from build123d import *

# Parameters (mm, degrees)
BOSS_EXTRUDE1_DEPTH = 5
SKETCH2_W           = 20
SKETCH2_H           = 6
SKETCH2_R           = 1.5
BOSS_EXTRUDE2_DEPTH = 2
SKETCH3_W           = 60
SKETCH3_H           = 6
BOSS_EXTRUDE3_DEPTH = 2


with BuildPart() as part:
    # Sketch1 → Boss-Extrude1 (new, symmetric)
    with BuildSketch(Plane.XY):
        Polygon((-14.216216216, 5.673798061), (-14.216216216, 15.673798061), (-16.216216216, 15.673798061), (-16.216216216, 3.673798061), (3.783783784, 3.673798061), (3.783783784, -6.326201939), (5.783783784, -6.326201939), (5.783783784, 5.673798061), align=None)
    extrude(amount=BOSS_EXTRUDE1_DEPTH, both=True)

    # Sketch2 → Boss-Extrude2 (add)
    with BuildSketch(Plane(origin=(5.783783784, 0, 0), x_dir=(0, 0, -1), z_dir=(1, 0, 0))):
        with Locations((0, -3.326201939)):
            Rectangle(SKETCH2_W, SKETCH2_H)
        with Locations((-7, -3.326201939)):
            Circle(SKETCH2_R, mode=Mode.SUBTRACT)
        with Locations((7, -3.326201939)):
            Circle(SKETCH2_R, mode=Mode.SUBTRACT)
    extrude(amount=-BOSS_EXTRUDE2_DEPTH)

    # Sketch3 → Boss-Extrude3 (add)
    with BuildSketch(Plane.ZY.offset(16.216216216)):
        with Locations((0, 12.673798061)):
            Rectangle(SKETCH3_W, SKETCH3_H)
    extrude(amount=-BOSS_EXTRUDE3_DEPTH)


solid = part.part
Geometry: final body of the model. Coordinates: model frame, mm. A direction names the side the tool comes from. Coordinates: 2 decimals unless noted, no trailing zeros. Order: outer loops, then holes, each group sorted by start corner. A loop starts at its lowest first (then second) coordinate and runs counter-clockwise, first axis right, second up.
(1) Material intervals for probe 1 along Z at (x, y) = (4, -3.25); probe 2 along Y at (x, z) = (4.95, 7); probe 3 along X at (y, z) = (11, -5), sorted ascending.
(2) Draft query along Z for faces 6 (the face through (5.784, -2, 0)), 7 (the face through (4.798, -2.312, 8.106)), 8 (the face through (-15, 13, 30)). Return one class per face: pulls with the +Z half, pulls with the -Z half, needs draft (parallel to the pull), parting line crosses it, or undercut.
(3) Section query C-C (x = -7). Return the cut outline in (y, z).
(4) Access query for faces 1 (the face through (5, -0.326, 8)), 2 (the face through (-4, 5.674, 0)), 3 (the face through (5, -0.326, -7)), 4 (the face through (-6, 5, -5)), 5 (the face through (3.784, -1, 0)). Directions: +Z, -Z, +X, -X, +Y, -Y. A direction counts if a zero-diameter tool reaches every point of the face in a straight line with its end or side. Return the directions, or none.
(5) First-contact query: pin 1 (0.6 mm diameter, centred on x = 4.5, y = -4.5, fed in from -Z); pin 2 (8 mm diameter, centred on x = -5.5, z = 0, fed in from +Y); pin 3 (8 mm diameter, centred on y = -3, z = -4, fed in from -X); pin 4 (2.5 mm diameter, centred on y = -3.33, z = 7, fed in from -X). Flat tips, straight axial feed; report the tip coordinate or a pass-through.
(6) Section query A-A (z = 7). Return the cut outline in (x, y), plus the area to 3 significant figures.
(7) Section query B-B (y = 11). Return the cut outline in (x, z).
Solution:
1. probe 1: z = -10 to -8.5, -5.5 to 5.5, 8.5 to 10
1. probe 2: y = -6.33 to -4.83, -1.83 to -0.33
1. probe 3: x = -16.22 to -14.22
2. face 6: needs draft
2. face 7: undercut
2. face 8: pulls with the +Z half
3. outline: (3.67, -5) - (5.67, -5) - (5.67, 5) - (3.67, 5) - close
4. face 1: +Z, +X, -X, +Y
4. face 2: +Z, -Z, +X, +Y
4. face 3: -Z, +X, -X, +Y
4. face 4: -Z, +X, -X
4. face 5: +Z, -Z, -X, -Y
5. pin 1: stops at z = -10
5. pin 2: stops at y = 5.67
5. pin 3: stops at x = 3.78
5. pin 4: passes through
6. outline: (-16.22, 9.67) - (-14.22, 9.67) - (-14.22, 15.67) - (-16.22, 15.67) - close; (3.78, -6.33) - (5.78, -6.33) - (5.78, -4.83) - (3.78, -4.83) - close; (3.78, -1.83) - (5.78, -1.83) - (5.78, -0.33) - (3.78, -0.33) - close
6. area: 18.0 mm2
7. outline: (-16.22, -30) - (-14.22, -30) - (-14.22, 30) - (-16.22, 30) - close
